Source: CAD feature listing. Evaluate the final solid. Frame: model axes, mm. A direction names the side the tool comes from. Round coordinates to 2 decimals unless told otherwise and drop trailing zeros. Loops run counter-clockwise (first coordinate to the right, second up) from the corner with the lowest first, then second, coordinate; pieces in that order, holes last.
Item 1: First-contact query: P1, Ø1, axis at y = 28.5, z = -2, coming from the +X side; P2, Ø1.5, axis at x = -0.5, y = 30.5, coming from the -Z side (3 decimals); P3, Ø1.5, axis at y = 34, z = -3, coming from the -X side. Flat tips, straight axial feed; report the tip coordinate or a pass-through.
Item 2: Ray query, L1, parallel to Y at x = 0, z = 3; L2, parallel to Y at x = 4.75, z = 0.5; L3, parallel to Z at x = -2.5, y = 36 (3 decimals). Return the intervals inside material, ascending.
Item 3: Section query B-B on z = 0. Return loops of the section in (x, y) (3 decimals), then the cut area to 3 significant figures.
Item 4: Section query A-A on x = 0. Return loops of the section in (y, z) (3 decimals), then the cut area to 3 significant figures.
Item 5: Access query for faces 1 (the cylindrical face through (2, 5, 0)), 2 (the flat face through (0, 0, 0)). Directions: +Z, -Z, +X, -X, +Y, -Y. A direction counts if a zero-diameter tool reaches every point of the face in a straight line with its end or side. Return the directions, or none.
Item 6: Section query C-C on y = 8. Return loops of the section in (x, z).
Item 7: Section query D-D on y = 37.5. Return loops of the section in (x, z).
Item 8: Pull-direction query (X, two-part tool) for faces 3 (the flat face through (3.3, 37, -0.1)), 4 (the cylindrical face through (4.88, 39.03, 1.08)); classes: released by +X, released by -X, zero draft, split by the parting line, or undercut.
```python
from build123d import *


with BuildPart() as part:
    # Screw Profile Sketch → Screw Body Revolve (revolve)
    with BuildSketch(Plane.XY, mode=Mode.PRIVATE) as screw_body_revolve_sk:
        Polygon((0, 0), (-2, 0), (-2, 10), (-3.125, 10), (-3.125, 37), (-5, 37), (-5, 41), (0, 41), align=None)
    revolve(screw_body_revolve_sk.sketch.rotate(Axis((0, 0, 0), (0, 1, 0)), 270), axis=Axis((0, 0, 0), (0, 1, 0)))


solid = part.part
```
Data:
1. P1: stops at x = 2.74
1. P2: stops at z = -3.125
1. P3: stops at x = -2.17
2. L1: y = 10 to 41
2. L2: y = 37 to 41
2. L3: z = -1.875 to 1.875
3. outline: (-5, 37) - (-3.125, 37) - (-3.125, 10) - (-2, 10) - (-2, 0) - (2, 0) - (2, 10) - (3.125, 10) - (3.125, 37) - (5, 37) - (5, 41) - (-5, 41) - close
3. area: 249 mm2
4. outline: (0, -2) - (10, -2) - (10, -3.125) - (37, -3.125) - (37, -5) - (41, -5) - (41, 5) - (37, 5) - (37, 3.125) - (10, 3.125) - (10, 2) - (0, 2) - close
4. area: 249 mm2
5. face 1: -Y
5. face 2: +Z, -Z, +X, -X, -Y
6. outline: circle Ø4 at (0, 0)
7. outline: circle Ø10 at (0, 0)
8. face 3: zero draft
8. face 4: split by the parting line
